Part model, mm, in its own coordinate system. Coordinates: 2 decimals unless noted, no trailing zeros. Write each loop counter-clockwise with the first axis right and the second up, starting at its lowest first coordinate (ties: lowest second). Pieces come first, ordered by that corner, then holes. Notation, with made-up numbers: (19.5, -18) -> (65.5, -18) arc R3 ccw to (65.5, -14) -> close; hole circle Ø11 at (-36, 10.25). An arc over 180 degrees is marked (long way). Write item = value, one per line.
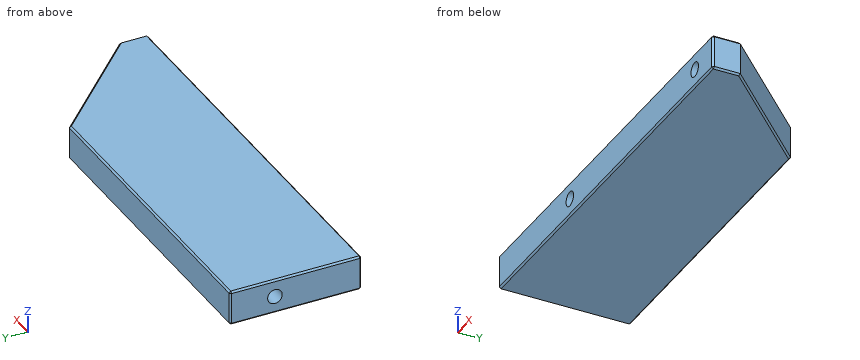
from build123d import *

# Parameters (mm, degrees)
SKETCH_1_W             = 120
SKETCH_1_H             = 38
EXTRUDE_1_DEPTH        = 10
CHAMFER_1_SIZE         = 30
HOLE_WIZARD_M5_1_D     = 4.2
HOLE_WIZARD_M5_1_DEPTH = 12.4
HOLE_WIZARD_M5_1_TIP   = 1.2618073
HOLE_WIZARD_M5_2_D     = 4.2
HOLE_WIZARD_M5_2_DEPTH = 12.4
HOLE_WIZARD_M5_2_TIP   = 1.2618073
CHAMFER_2_SIZE         = 0.5


with BuildPart() as part:
    # 草图1 → 凸台-拉伸1 (new body)
    with BuildSketch(Plane.XY):
        Rectangle(SKETCH_1_W, SKETCH_1_H)
    extrude(amount=EXTRUDE_1_DEPTH)

    # 倒角1
    chamfer_1_edges = [part.edges().sort_by_distance(p)[0] for p in [
        (60, 19, 5),
    ]]
    chamfer(chamfer_1_edges, length=CHAMFER_1_SIZE)

    # M5 螺纹孔1
    with Locations(Plane.ZY.offset(60)):
        with Locations((5, 6)):
            Hole(HOLE_WIZARD_M5_1_D / 2, depth=HOLE_WIZARD_M5_1_DEPTH)
            with Locations((0, 0, -(HOLE_WIZARD_M5_1_DEPTH + HOLE_WIZARD_M5_1_TIP / 2))):  # 118° drill point
                Cone(0, HOLE_WIZARD_M5_1_D / 2, HOLE_WIZARD_M5_1_TIP, mode=Mode.SUBTRACT)

    # M5 螺纹孔2
    with Locations(Plane(origin=(0, -19, 0), x_dir=(-1, 0, 0), z_dir=(0, -1, 0))):
        with Locations((-50, -5), (20, -5)):
            Hole(HOLE_WIZARD_M5_2_D / 2, depth=HOLE_WIZARD_M5_2_DEPTH)
            with Locations((0, 0, -(HOLE_WIZARD_M5_2_DEPTH + HOLE_WIZARD_M5_2_TIP / 2))):  # 118° drill point
                Cone(0, HOLE_WIZARD_M5_2_D / 2, HOLE_WIZARD_M5_2_TIP, mode=Mode.SUBTRACT)

    # 倒角2
    chamfer_2_edges = [part.edges().sort_by_distance(p)[0] for p in [
        (-60, 0, 10),
        (-15, 19, 0),
        (-15, 19, 10),
        (45, 4, 0),
        (45, 4, 10),
        (0, -19, 10),
        (60, -15, 10),
        (0, -19, 0),
        (-60, 0, 0),
        (60, -15, 0),
        (60, -19, 5),
        (-60, -19, 5),
        (-60, 19, 5),
    ]]
    chamfer(chamfer_2_edges, length=CHAMFER_2_SIZE)


solid = part.part
Q1. Pin check, flat tips, straight feed: pin 1 (2 mm diameter, centred on y = 15, z = 2, fed in from +X); pin 2 (2 mm diameter, centred on y = 3.5, z = 8.5, fed in from +X); pin 3 (5 mm diameter, centred on x = 50, z = 5, fed in from +Y). Stop position of each tip, or through.
Model answer:
pin_1 = 35
pin_2 = 46.5
pin_3 = 1.5
Q2. Saw through at B-B on y = 12. Give the cut face in (x, z), and give its area (3 significant figures).
Model answer:
outline = (-60, 0.5) -> (-59.5, 0) -> (36.29, 0) -> (37, 0.5) -> (37, 9.5) -> (36.29, 10) -> (-59.5, 10) -> (-60, 9.5) -> close
area = 969 mm²
Q3. Probe line 1 (Y direction, x = -53, z = 5); line 2 (X direction, y = -17, z = 6); line 3 (Z direction, x = -56.75, y = 6). List the from-to ranges inside material, lowest first. Write a range as from..to.
Model answer:
line_1 = -19..3.9, 8.1..19
line_2 = -60..-21.85, -18.15..48.15, 51.85..60
line_3 = 0..2.9, 7.1..10
Q4. Saw through at A-A on y = -4. Give the cut face in (x, z).
Model answer:
outline = (-60, 0.5) -> (-59.5, 0) -> (52.29, 0) -> (53, 0.5) -> (53, 9.5) -> (52.29, 10) -> (-59.5, 10) -> (-60, 9.5) -> close
